```python
from build123d import *

# Parameters (mm, degrees)
SKETCH_1_W                = 65
SKETCH_1_H                = 85
EXTRUDE_1_DEPTH           = 35
SKETCH_2_W                = 109.971307268
SKETCH_2_H                = 65
CUT_EXTRUDE_1_DEPTH       = 27
SKETCH_3_R                = 19.25
CUT_EXTRUDE_2_DEPTH       = 64.933559263
HOLE_WIZARD_M4_1_D        = 3.3
HOLE_WIZARD_M3_1_D        = 2.5
HOLE_WIZARD_M3_1_DEPTH    = 12.5
HOLE_WIZARD_M3_1_TIP      = 0.751075774
CUT_EXTRUDE_3_DEPTH       = 15
HOLE_WIZARD_1_D           = 4.5
HOLE_WIZARD_1_CBORE_D     = 8
HOLE_WIZARD_1_CBORE_DEPTH = 20
HOLE_WIZARD_M3_3_D        = 2.5
HOLE_WIZARD_M3_3_DEPTH    = 9.5
HOLE_WIZARD_M3_3_TIP      = 0.751075774


with BuildPart() as part:
    # 草图1 → 凸台-拉伸1 (new body)
    with BuildSketch(Plane(origin=(0, 0, 0), x_dir=(1, 0, 0), z_dir=(0, 1, 0))):
        Rectangle(SKETCH_1_W, SKETCH_1_H)
    extrude(amount=EXTRUDE_1_DEPTH)

    # 草图2 → 切除-拉伸1 (cut)
    with BuildSketch(Plane.XZ):
        Rectangle(SKETCH_2_W, SKETCH_2_H)
    extrude(amount=-CUT_EXTRUDE_1_DEPTH, mode=Mode.SUBTRACT)

    # 草图3 → 切除-拉伸2 (cut, through all)
    with BuildSketch(Plane(origin=(0, 35, 0), x_dir=(1, 0, 0), z_dir=(0, 1, 0))):
        with Locations(Location((0, 0, 0), (0, 0, 270))):
            Circle(SKETCH_3_R)
    extrude(amount=-CUT_EXTRUDE_2_DEPTH, mode=Mode.SUBTRACT)

    # M4 螺纹孔1 (through all)
    with Locations(Plane(origin=(0, 35, 0), x_dir=(1, 0, 0), z_dir=(0, 1, 0))):
        with Locations((-23.57, 23.57), (23.57, 23.57), (-23.57, -23.57), (23.57, -23.57)):
            Hole(HOLE_WIZARD_M4_1_D / 2)

    # M3 螺纹孔1
    with Locations(Plane.ZY.offset(32.5)):
        with Locations((7.5, 31), (-7.5, 31)):
            Hole(HOLE_WIZARD_M3_1_D / 2, depth=HOLE_WIZARD_M3_1_DEPTH)
            with Locations((0, 0, -(HOLE_WIZARD_M3_1_DEPTH + HOLE_WIZARD_M3_1_TIP / 2))):  # 118° drill point
                Cone(0, HOLE_WIZARD_M3_1_D / 2, HOLE_WIZARD_M3_1_TIP, mode=Mode.SUBTRACT)

    # 草图10 → 切除-拉伸3 (cut)
    with BuildSketch(Plane(origin=(0, 0, -42.5), x_dir=(-1, 0, 0), z_dir=(0, 0, -1))):
        with BuildLine():
            Line((-27.5, 13.5), (-37.5, 13.5))
            ThreePointArc((-37.5, 13.5), (-41.5, 17.5), (-37.5, 21.5))
            Line((-37.5, 21.5), (-27.5, 21.5))
            ThreePointArc((-27.5, 21.5), (-23.5, 17.5), (-27.5, 13.5))
        make_face()
    extrude(amount=-CUT_EXTRUDE_3_DEPTH, mode=Mode.SUBTRACT)

    # 打孔尺寸(%根据)开槽圆柱头螺钉的类型1 (through all)
    with Locations(Plane(origin=(0, 35, 0), x_dir=(1, 0, 0), z_dir=(0, 1, 0))):
        with Locations((-17.5, 37.5), (17.5, 37.5), (-17.5, -37.5), (17.5, -37.5)):
            CounterBoreHole(HOLE_WIZARD_1_D / 2, HOLE_WIZARD_1_CBORE_D / 2, HOLE_WIZARD_1_CBORE_DEPTH)

    # M3 螺纹孔3
    with Locations(Plane(origin=(0, 35, 0), x_dir=(1, 0, 0), z_dir=(0, 1, 0))):
        with Locations((-24.99999811, 32.299994492), (-24.99999811, 39.299998272)):
            Hole(HOLE_WIZARD_M3_3_D / 2, depth=HOLE_WIZARD_M3_3_DEPTH)
            with Locations((0, 0, -(HOLE_WIZARD_M3_3_DEPTH + HOLE_WIZARD_M3_3_TIP / 2))):  # 118° drill point
                Cone(0, HOLE_WIZARD_M3_3_D / 2, HOLE_WIZARD_M3_3_TIP, mode=Mode.SUBTRACT)


solid = part.part
```
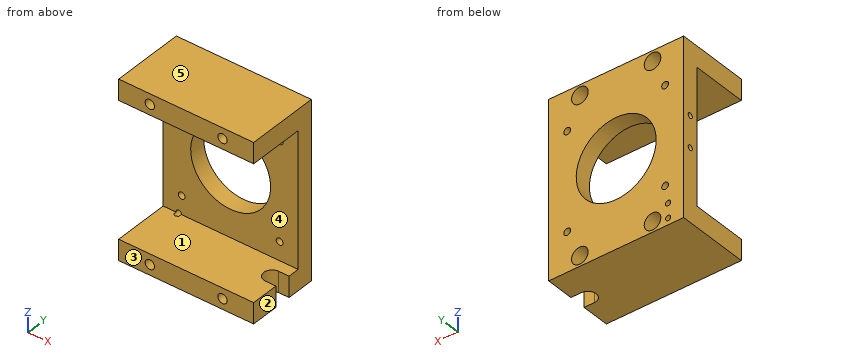
The model under review builds one solid part; all positions refer to its coordinate system, in mm. Face numbers are marked on the shaded views. A direction names the side the tool comes from. Round coordinates to 2 decimals unless told otherwise and drop trailing zeros. Write each loop counter-clockwise with the first axis right and the second up, starting at its lowest first coordinate (ties: lowest second). Pieces come first, ordered by that corner, then holes.
(1) Mouldability with a two-part tool opening along Z and no side actions: class the marked faces 3, 4 and 5 as +Z half, -Z half, draft (parallel to the pull), parting line (faces both ways), or undercut.
(2) Wall thickness on L1, parallel to Z at x = -17.5, y = 7.75; L2, parallel to Z at x = -23.57, y = 33; L3, parallel to X at y = 33, z = -23.57: over which ranges is each line inside the solid? List them lowest first.
(3) We need section C-C on x = 18. Give the boundary of the cut face in (y, z), and give its area (3 significant figures).
(4) Machinability: for the marked faces 1 and 2, which of the approach directions +Z, -Z, +X, -X, +Y, -Y give a long, thin tool a straight path to every point of the face, cutting with its end or side? Answer none if there is none.
(5) We need section A-A on y = 17.5. Give the boundary of the cut face in (x, z).
(6) Insertion check: pin 1 (1 mm diameter, centred on y = 21.5, z = -31.5, fed in from -X); pin 2 (1 mm diameter, centred on x = 24.5, z = 22, fed in from -Y); pin 3 (5 mm diameter, centred on x = -17.5, z = 37.5, fed in from +Y). Each pin has a flat end and moves straight along its axis. Give the tip position at first contact, or say it passes through.
(7) We need section B-B on z = -23.57. Give the boundary of the cut face in (x, y), and give its area (3 significant figures).
(8) We need section D-D on z = 0. Give the boundary of the cut face in (x, y), and give its area (3 significant figures).
Findings below:
1. face 3: draft
1. face 4: undercut
1. face 5: +Z half
2. L1: z = -42.5 to -39.75, -35.25 to -32.5, 32.5 to 35.25, 39.75 to 42.5
2. L2: z = -42.5 to -25.22, -21.92 to 21.92, 25.22 to 42.5
2. L3: x = -32.5 to -25.22, -21.92 to 21.92, 25.22 to 32.5
3. outline: (0, -42.5) - (35, -42.5) - (35, -41.47) - (15, -41.47) - (15, -39.69) - (0, -39.69) - close; (0, -35.31) - (15, -35.31) - (15, -33.53) - (35, -33.53) - (35, -6.82) - (27, -6.82) - (27, -32.5) - (0, -32.5) - close; (0, 32.5) - (27, 32.5) - (27, 6.82) - (35, 6.82) - (35, 33.53) - (15, 33.53) - (15, 35.31) - (0, 35.31) - close; (0, 39.69) - (15, 39.69) - (15, 41.47) - (35, 41.47) - (35, 42.5) - (0, 42.5) - close
3. area: 662 mm2
4. face 1: +X, -X, -Y
4. face 2: +Z, -Z, +X, +Y, -Y
5. outline: (-32.5, -42.5) - (23.5, -42.5) - (23.5, -32.5) - (-32.5, -32.5) - close; (-32.5, 32.5) - (32.5, 32.5) - (32.5, 42.5) - (-32.5, 42.5) - close; hole circle Ø8 at (-17.5, -37.5); hole circle Ø8 at (-17.5, 37.5); hole circle Ø8 at (17.5, -37.5); hole circle Ø8 at (17.5, 37.5)
6. pin 1: passes through
6. pin 2: stops at y = 27
6. pin 3: stops at y = 15
7. outline: (-32.5, 27) - (-25.22, 27) - (-25.22, 35) - (-32.5, 35) - close; (-21.92, 27) - (21.92, 27) - (21.92, 35) - (-21.92, 35) - close; (25.22, 27) - (32.5, 27) - (32.5, 35) - (25.22, 35) - close
7. area: 467 mm2
8. outline: (-32.5, 27) - (-19.25, 27) - (-19.25, 35) - (-32.5, 35) - close; (19.25, 27) - (32.5, 27) - (32.5, 35) - (19.25, 35) - close
8. area: 212 mm2
